The figure shows three views and two pictorial views of one solid part (mm, origin at its lowest corner). Answer the questions. Round coordinates to 2 decimals unless told otherwise and drop trailing zeros. Order: outer loops, then holes, each group sorted by start corner. A loop starts at its lowest first (then second) coordinate and runs counter-clockwise, first axis right, second up. Notation, with made-up numbers: (32, 81.5) - (70, 81.5) arc R22 ccw to (70, 93.5) - close; hole circle Ø9 at (83.25, -16). An arc over 180 degrees is marked (long way). One line per item, written item: value. Start each with the question number.
1. Section A-A, the plane x = 50 is taken. Give the vertices of the cut face in (y, z), then the cut area to 3 significant figures.
2. Straight lines are drawn through the part: line 1 (X direction, y = 3.5, z = 50); line 2 (Z direction, x = 14.5, y = 3.5) (1 decimal); line 3 (X direction, y = 6.25, z = 32). For each, find the intervals that lie inside material, in ascending order.
3. Section C-C, the plane y = 3.25 is taken. Give the vertices of the cut face in (x, z), then the cut area to 3 significant figures.
4. A flat-ended cylindrical pin translates along its axis: P1, Ø6.5, axis at x = 86.77, z = 13.23, coming from the -Y side. Find the tip coordinate at first contact, or state that the pin passes through.
5. Section B-B, the plane z = 50 is taken. Give the vertices of the cut face in (x, y), then the cut area to 3 significant figures.
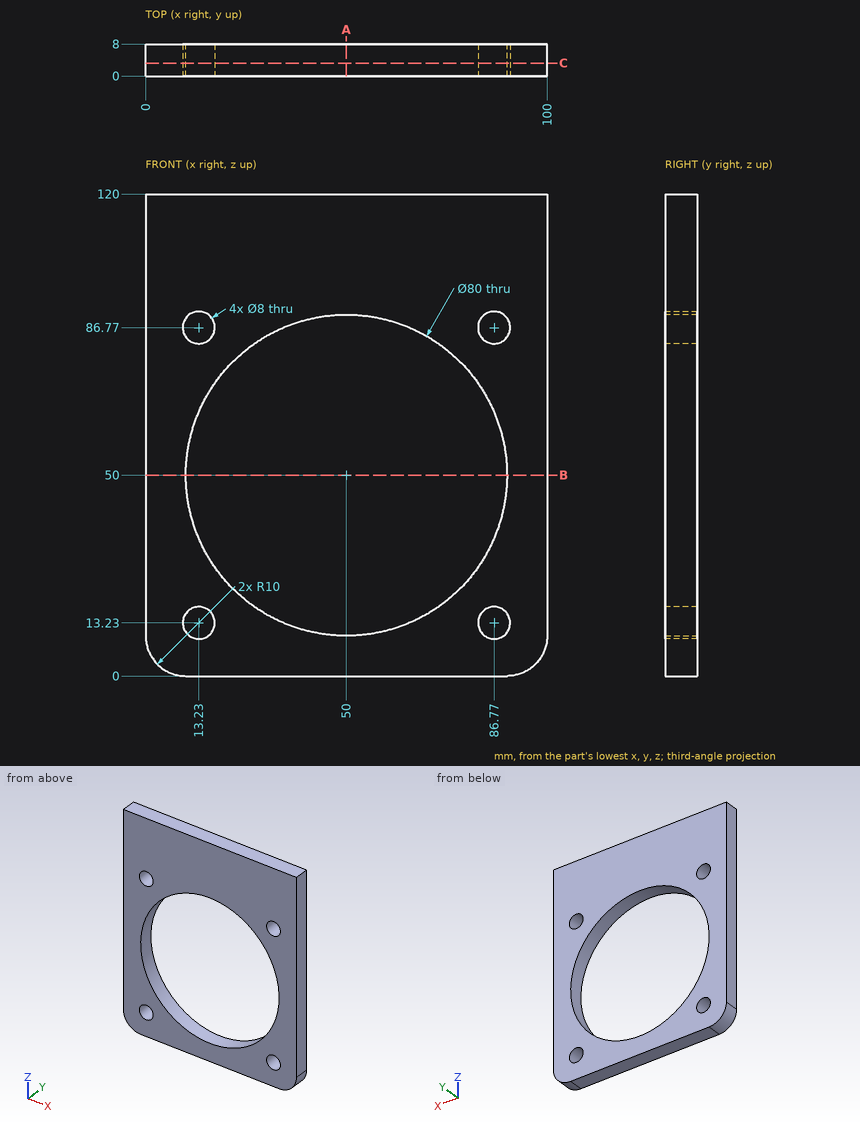
Answer list:
1. outline: (0, 0) - (8, 0) - (8, 10) - (0, 10) - close; (0, 90) - (8, 90) - (8, 120) - (0, 120) - close
1. area: 320 mm²
2. line 1: x = 0 to 10, 90 to 100
2. line 2: z = 0 to 9.4, 17 to 31.6, 68.4 to 83, 90.6 to 120
2. line 3: x = 0 to 14.28, 85.72 to 100
3. outline: (0, 10) arc R10 ccw to (10, 0) - (90, 0) arc R10 ccw to (100, 10) - (100, 120) - (0, 120) - close; hole circle Ø8 at (13.23, 13.23); hole circle Ø8 at (13.23, 86.77); hole circle Ø80 at (50, 50); hole circle Ø8 at (86.77, 13.23); hole circle Ø8 at (86.77, 86.77)
3. area: 6,730 mm²
4. P1: passes through
5. outline: (0, 0) - (10, 0) - (10, 8) - (0, 8) - close; (90, 0) - (100, 0) - (100, 8) - (90, 8) - close
5. area: 160 mm²
